from build123d import *

# Parameters (mm, degrees)
SKETCH_1_R          = 22.5
EXTRUDE_1_DEPTH     = 65
SKETCH_2_R          = 5
EXTRUDE_2_DEPTH     = 25
SKETCH_3_W          = 22.5
SKETCH_3_H          = 55
EXTRUDE_3_DEPTH     = 5
SKETCH_4_W          = 22.5
SKETCH_4_H          = 55
EXTRUDE_4_DEPTH     = 5
CUT_EXTRUDE_1_DEPTH = 55
SKETCH_6_R          = 2.5
CUT_EXTRUDE_2_DEPTH = 60


with BuildPart() as part:
    # 草图1 → 凸台-拉伸1 (new body)
    with BuildSketch(Plane.XY):
        Circle(SKETCH_1_R)
    extrude(amount=EXTRUDE_1_DEPTH)

    # 草图2 → 凸台-拉伸2 (add)
    with BuildSketch(Plane.XY.offset(65)):
        Circle(SKETCH_2_R)
    extrude(amount=EXTRUDE_2_DEPTH)

    # 草图3 → 凸台-拉伸3 (add)
    with BuildSketch(Plane(origin=(0, 22.5, 0), x_dir=(-1, 0, 0), z_dir=(0, 1, 0))):
        with Locations((-11.25, 27.5)):
            Rectangle(SKETCH_3_W, SKETCH_3_H)
    extrude(amount=-EXTRUDE_3_DEPTH)

    # 草图4 → 凸台-拉伸4 (add)
    with BuildSketch(Plane(origin=(0, -22.5, 0), x_dir=(-1, 0, 0), z_dir=(0, 1, 0))):
        with Locations((-11.25, 27.5)):
            Rectangle(SKETCH_4_W, SKETCH_4_H)
    extrude(amount=EXTRUDE_4_DEPTH)

    # 草图5 → 切除-拉伸1 (cut)
    with BuildSketch(Plane(origin=(0, 0, 0), x_dir=(-1, 0, 0), z_dir=(0, 0, -1))):
        with BuildLine():
            Line((-14.142135624, -17.5), (0, -17.5))
            Line((0, -17.5), (0, 17.5))
            Line((0, 17.5), (-14.142135624, 17.5))
            ThreePointArc((-14.142135624, 17.5), (-22.5, 0), (-14.142135624, -17.5))
        make_face()
    extrude(amount=-CUT_EXTRUDE_1_DEPTH, mode=Mode.SUBTRACT)

    # 草图6 → 切除-拉伸2 (cut)
    with BuildSketch(Plane.XZ.offset(22.5)):
        with Locations(Location((17.5, 5, 0), (0, 0, 270))):
            Circle(SKETCH_6_R)
        with Locations(Location((17.5, 45, 0), (0, 0, 270))):
            Circle(SKETCH_6_R)
    extrude(amount=-CUT_EXTRUDE_2_DEPTH, mode=Mode.SUBTRACT)


solid = part.part
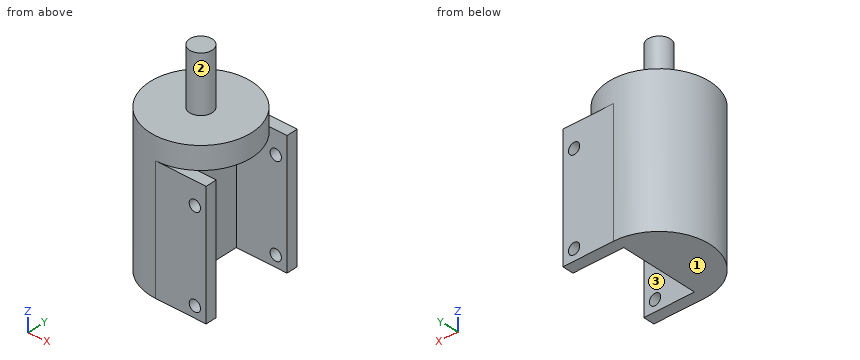
Work out the finished part from the listing and answer in its coordinate system (mm). Face numbers are marked on the shaded views. A direction names the side the tool comes from. Give positions to 0.01 mm unless a question says otherwise; leave off trailing zeros. Write each loop counter-clockwise with the first axis right and the second up, starting at its lowest first coordinate (ties: lowest second). Pieces come first, ordered by that corner, then holes. Notation, with made-up numbers: (-25.5, 31) - (-6.5, 31) arc R38 cw to (-6.5, 70) - close; hole circle Ø9 at (-22.5, 26). An arc over 180 degrees is marked (long way). One line per item, written item: value. Start each with the question number.
1. Find section B-B (x = 19). Write down the section's boundary in (y, z), then the cut area to 3 significant figures.
2. Given pin 1 (12 mm diameter, centred on x = 18, z = 67.5, fed in from +Y); pin 2 (5 mm diameter, centred on y = -6.5, z = 32.5, fed in from +X); pin 3 (10 mm diameter, centred on x = -17, z = 43, fed in from -Y), each flat-ended and moving along its own axis, determine where each tip first touches the part or whether it passes through.
3. Find section D-D (y = -16). Write down the section's boundary in (x, z).
4. Find section C-C (z = 21). Write down the section's boundary in (x, y).
5. Find section A-A (z = 5). Write down the section's boundary in (x, y).
6. Consider probe 1 along Y at (x, z) = (8, 45.5); probe 2 along Z at (x, y) = (17, -20); probe 3 along Z at (x, y) = (4, 2). Determine where each line is inside the solid, lowest interval first.
7. For the marked faces 1, 2 and 3, determine the directions among +Z, -Z, +X, -X, +Y, -Y from which every point of the face is accessible in a straight line to the end or side of a thin tool.
Geometry results:
1. outline: (-22.5, 0) - (-17.5, 0) - (-17.5, 3) - (-22.5, 3) - close; (-22.5, 7) - (-17.5, 7) - (-17.5, 43) - (-22.5, 43) - close; (-22.5, 47) - (-17.5, 47) - (-17.5, 55) - (-22.5, 55) - close; (-12.05, 55) - (12.05, 55) - (12.05, 65) - (-12.05, 65) - close; (17.5, 0) - (22.5, 0) - (22.5, 3) - (17.5, 3) - close; (17.5, 7) - (22.5, 7) - (22.5, 43) - (17.5, 43) - close; (17.5, 47) - (22.5, 47) - (22.5, 55) - (17.5, 55) - close
1. area: 711 mm2
2. pin 1: y = 18.68
2. pin 2: x = 0
2. pin 3: y = -19.03
3. outline: (-15.82, 0) - (0, 0) - (0, 55) - (15.82, 55) - (15.82, 65) - (-15.82, 65) - close
4. outline: (0, -22.5) - (22.5, -22.5) - (22.5, -17.5) - (0, -17.5) - (0, 17.5) - (22.5, 17.5) - (22.5, 22.5) - (0, 22.5) arc R22.5 ccw to start
5. outline: (0, -22.5) - (15, -22.5) - (15, -17.5) - (0, -17.5) - (0, 17.5) - (15, 17.5) - (15, 22.5) - (0, 22.5) arc R22.5 ccw to start; (20, -22.5) - (22.5, -22.5) - (22.5, -17.5) - (20, -17.5) - close; (20, 17.5) - (22.5, 17.5) - (22.5, 22.5) - (20, 22.5) - close
6. probe 1: -22.5 to -17.5, 17.5 to 22.5
6. probe 2: 0 to 2.55, 7.45 to 42.55, 47.45 to 55
6. probe 3: 55 to 90
7. face 1: -Z, +X, -X, +Y, -Y
7. face 2: +Z
7. face 3: -Z, +X
